For this review, take the finished solid that the model builds, in its own axes (mm). Give positions to 0.01 mm unless a question says otherwise; leave off trailing zeros. Order: outer loops, then holes, each group sorted by start corner. A loop starts at its lowest first (then second) coordinate and runs counter-clockwise, first axis right, second up.
Item 1: For P1, Ø3, axis at x = 49, y = 1.5, coming from the -Z side, flat-tipped, find the tip position at first contact; note if it passes through.
Item 2: Consider section A-A (y = 0). Give the boundary of the cut face in (x, z) (3 decimals), plus the area to 3 significant figures.
Item 3: The part is to be moulded in two halves that separate along Y. For faces 1 (the flat face through (2, 0, 2.5)), 2 (the cylindrical face through (170.654, 1.502, 1.232)), 3 (the cylindrical face through (175.883, 0.22, 1.232)), say which applies: released by +Y, released by -Y, zero draft, split by the parting line, or undercut.
Item 4: Consider section B-B (z = 0.4). Give the boundary of the cut face in (x, y) (3 decimals).
Item 5: For probe 1 along X at (y, z) = (-0.25, 1); probe 2 along X at (y, z) = (-3.75, 1.75); probe 3 along X at (y, z) = (7.25, 0.35), list the stretches that pass through material, from the lowest coordinate up.
```python
from build123d import *

# Parameters (mm, degrees)
SKETCH1_R           = 5
BOSS_EXTRUDE1_DEPTH = 2.5


with BuildPart() as part:
    # Sketch1 → Boss-Extrude1 (new body)
    with BuildSketch(Plane.XY):
        with BuildLine():
            Line((-165.885, 10), (165.885, 10))
            ThreePointArc((165.885, 10), (175.885, 0), (165.885, -10))
            Line((165.885, -10), (-165.885, -10))
            ThreePointArc((-165.885, -10), (-175.885, 0), (-165.885, 10))
        make_face()
        with Locations((-165.885, 0)):
            Circle(SKETCH1_R, mode=Mode.SUBTRACT)
        with Locations((165.885, 0)):
            Circle(SKETCH1_R, mode=Mode.SUBTRACT)
    extrude(amount=BOSS_EXTRUDE1_DEPTH)


solid = part.part
```
Resolved:
1. P1: stops at z = 0
2. outline: (-175.885, 0) - (-170.885, 0) - (-170.885, 2.5) - (-175.885, 2.5) - close; (-160.885, 0) - (160.885, 0) - (160.885, 2.5) - (-160.885, 2.5) - close; (170.885, 0) - (175.885, 0) - (175.885, 2.5) - (170.885, 2.5) - close
2. area: 829 mm2
3. face 1: zero draft
3. face 2: undercut
3. face 3: split by the parting line
4. outline: (-165.885, -10) - (165.885, -10) arc R10 ccw to (165.885, 10) - (-165.885, 10) arc R10 ccw to start; hole circle Ø10 at (-165.885, 0); hole circle Ø10 at (165.885, 0)
5. probe 1: x = -175.88 to -170.88, -160.89 to 160.89, 170.88 to 175.88
5. probe 2: x = -175.16 to -169.19, -162.58 to 162.58, 169.19 to 175.16
5. probe 3: x = -172.77 to 172.77
